Read the model definition and answer for the solid it produces. Units are mm, in the model's axes. Face numbers are marked on the shaded views. A direction names the side the tool comes from. Coordinates: 2 decimals unless noted, no trailing zeros. Loops run counter-clockwise (first coordinate to the right, second up) from the corner with the lowest first, then second, coordinate; pieces in that order, holes last. Notation, with made-up numbers: (47, 61) - (99, 61) arc R27 ccw to (99, 96) - close; hole circle Ø4 at (72.25, 24). An arc over 180 degrees is marked (long way). One line per question, with ' | ' between items. Start each with the question number.
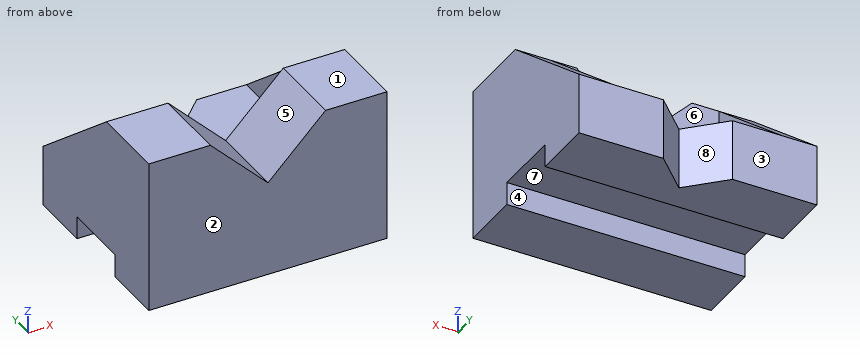
```python
from build123d import *

# Parameters (mm, degrees)
BASE_PROFILE_SKETCH_W = 124
BASE_PROFILE_SKETCH_H = 100
BASE_BLOCK_32_DEPTH   = 32
FRONT_NOTCH_SKETCH_W  = 12
FRONT_NOTCH_SKETCH_H  = 36
FRONT_NOTCH_CUT_DEPTH = 124
UPRIGHT_WALL_SKETCH_W = 124
UPRIGHT_WALL_SKETCH_H = 48
UPRIGHT_WALL_40_DEPTH = 40
WEDGE_A_18_DEPTH      = 18
WEDGE_B_18_DEPTH      = 18
V_NOTCH_CUT_DEPTH     = 40
SIDE_SLOT_CUT_DEPTH   = 40


with BuildPart() as part:
    # Base Profile Sketch → Base Block 32 (new body)
    with BuildSketch(Plane.XY):
        with Locations((62, -50)):
            Rectangle(BASE_PROFILE_SKETCH_W, BASE_PROFILE_SKETCH_H)
    extrude(amount=BASE_BLOCK_32_DEPTH)

    # Front Notch Sketch → Front Notch Cut (cut)
    with BuildSketch(Plane.ZY):
        with Locations((6, -50)):
            Rectangle(FRONT_NOTCH_SKETCH_W, FRONT_NOTCH_SKETCH_H)
    extrude(amount=-FRONT_NOTCH_CUT_DEPTH, mode=Mode.SUBTRACT)

    # Upright Wall Sketch → Upright Wall 40 (add)
    with BuildSketch(Plane.XZ.offset(100)):
        with Locations((62, 56)):
            Rectangle(UPRIGHT_WALL_SKETCH_W, UPRIGHT_WALL_SKETCH_H)
    extrude(amount=-UPRIGHT_WALL_40_DEPTH)

    # Wedge A Sketch → Wedge A 18 (add)
    with BuildSketch(Plane(origin=(124, 0, 0), x_dir=(0, 0, -1), z_dir=(1, 0, 0))):
        Polygon((-80, -60), (-32, 0), (-32, -60), align=None)
    extrude(amount=-WEDGE_A_18_DEPTH)

    # Wedge B Sketch → Wedge B 18 (add)
    with BuildSketch(Plane.ZY):
        Polygon((80, -60), (32, 0), (32, -60), align=None)
    extrude(amount=-WEDGE_B_18_DEPTH)

    # V Notch Sketch → V Notch Cut (cut)
    with BuildSketch(Plane(origin=(0, -60, 0), x_dir=(1, 0, 0), z_dir=(0, 1, 0))):
        Polygon((32, -80), (62, -80), (92, -80), (62, -50), align=None)
    extrude(amount=-V_NOTCH_CUT_DEPTH, mode=Mode.SUBTRACT)

    # Side Slot Sketch → Side Slot Cut (cut)
    with BuildSketch(Plane.XY.offset(32)):
        Polygon((80, 0), (62, 0), (44, 0), (62, -18), align=None)
    extrude(amount=-SIDE_SLOT_CUT_DEPTH, mode=Mode.SUBTRACT)


solid = part.part
```
1) The mould has two halves that part along Y. Classify the marked faces 1, 2, 3 and 4: released by +Y, released by -Y, zero draft, split by the parting line, or undercut.
2) Which of the six approach directions +Z, -Z, +X, -X, +Y, -Y give full straight-line access (tool end or side, diameter ignored) to the marked faces 5, 6, 7 and 8?
3) Find the intervals of material crossed by line 1 along X through (y, z) = (-9, 33); line 2 along Y through (x, z) = (17, 9.5); line 3 along Z through (x, y) = (71.5, -52.5), in increasing order. Write a range as from..to.
4) The part is cut by section D-D on z = 37. Write down the section's boundary in (x, y), and give its area (4 significant figures).
5) The part is cut by section B-B on y = -37. Write down the section's boundary in (x, z), and give its area (3 significant figures).
6) Given pin 1 Ø3 at (x, z) = (77.5, 22.5) entering from +Y; pin 2 Ø12 at (x, y) = (92.5, -12) entering from +Z; pin 3 Ø8 at (x, z) = (48.5, 8) entering from +Y, each flat-ended and moving along its own axis, determine where each tip first touches the part or whether it passes through.
7) The part is cut by section A-A on z = 6. Write down the section's boundary in (x, y), and give its area (3 significant figures).
8) The part is cut by section C-C on x = 73. Write down the section's boundary in (y, z), and give its area (3 significant figures).
Answer below:
1) face 1: zero draft | face 2: released by -Y | face 3: released by +Y | face 4: undercut
2) face 5: +Z, +Y, -Y | face 6: +Z, +Y | face 7: -Z, +X, -X | face 8: +Z, -Z, +Y
3) line 1: 0..18, 106..124 | line 2: -100..-68, -32..0 | line 3: 12..32
4) outline: (0, -100) - (124, -100) - (124, -6.25) - (106, -6.25) - (106, -60) - (18, -60) - (18, -6.25) - (0, -6.25) - close | area: 6,895 mm2
5) outline: (0, 12) - (124, 12) - (124, 61.6) - (106, 61.6) - (106, 32) - (18, 32) - (18, 61.6) - (0, 61.6) - close | area: 3,550 mm2
6) pin 1: y = -1 | pin 2: z = 32 | pin 3: y = -0.5
7) outline: (0, -100) - (124, -100) - (124, -68) - (0, -68) - close; (0, -32) - (124, -32) - (124, 0) - (80, 0) - (62, -18) - (44, 0) - (0, 0) - close | area: 7,610 mm2
8) outline: (-100, 0) - (-68, 0) - (-68, 12) - (-32, 12) - (-32, 0) - (-7, 0) - (-7, 32) - (-60, 32) - (-60, 61) - (-100, 61) - close | area: 3,700 mm2
